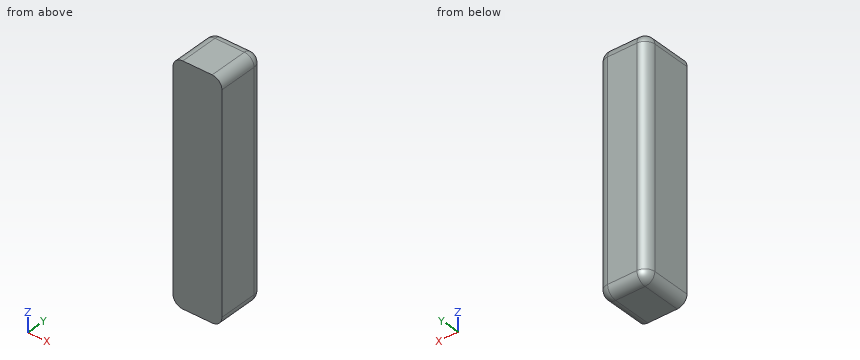
from build123d import *

# Parameters (mm, degrees)
SKETCH_1_W          = 50
SKETCH_1_H          = 50
EXTRUDE_2_DEPTH     = 240
EXTRUDE_3_DEPTH     = 5
FILLET_1_R          = 10
SKETCH_3_W          = 340
SKETCH_3_H          = 5
CUT_EXTRUDE_1_DEPTH = 59


with BuildPart() as part:
    # 草图1 → 凸台-拉伸2 (new body)
    with BuildSketch(Plane.XY):
        with Locations((25, 25)):
            Rectangle(SKETCH_1_W, SKETCH_1_H)
    extrude(amount=EXTRUDE_2_DEPTH)

    # 草图2 → 凸台-拉伸3 (add)
    with BuildSketch(Plane.XZ):
        Polygon((0, 240), (0, 290), (50, 290), (50, 0), (50, -50), (0, -50), align=None)
    extrude(amount=EXTRUDE_3_DEPTH)

    # 圆角1
    fillet_1_edges = [part.edges().sort_by_distance(p)[0] for p in [
        (25, 50, 240),
        (0, 25, 240),
        (50, 25, 240),
        (50, 50, 120),
        (50, 25, 0),
        (0, 25, 0),
        (25, 50, 0),
        (0, 50, 120),
    ]]
    fillet(fillet_1_edges, radius=FILLET_1_R)

    # 草图3 → 切除-拉伸1 (cut)
    with BuildSketch(Plane.ZY):
        with Locations((120, -2.5)):
            Rectangle(SKETCH_3_W, SKETCH_3_H)
    extrude(amount=-CUT_EXTRUDE_1_DEPTH, mode=Mode.SUBTRACT)


solid = part.part
Geometry check sheet. Reference: the model listing, model coordinates, mm. Give positions to 0.01 mm unless a question says otherwise; leave off trailing zeros. Order: outer loops, then holes, each group sorted by start corner. A loop starts at its lowest first (then second) coordinate and runs counter-clockwise, first axis right, second up.
1) Cross-section at A-A (z = 191.5). Record the boundary of the cut face in (x, y).
Results are:
outline: (0, 0) - (50, 0) - (50, 40) arc R10 ccw to (40, 50) - (10, 50) arc R10 ccw to (0, 40) - close
2) Gauge pin test, flat end, axial feed: pin 1 (1 mm diameter, centred on x = 8.5, y = 12.5, fed in from -Z). Record the tip position at first contact, or that the pin passes through.
Results are:
pin 1: stops at z = 0.05
3) Cross-section at C-C (x = 5). Record the boundary of the cut face in (y, z).
Results are:
outline: (0, 1.34) - (40, 1.34) arc R8.66 ccw to (48.66, 10) - (48.66, 230) arc R8.66 ccw to (40, 238.66) - (0, 238.66) - close
4) Material ranges on probe 1 along Z at (x, y) = (7, 39.5); probe 2 along Y at (x, z) = (4.5, 132.5); probe 3 along X at (y, z) = (41.5, 184.5), recorded low to high.
Results are:
probe 1: z = 0.46 to 239.54
probe 2: y = 0 to 48.35
probe 3: x = 0.11 to 49.89
5) Cross-section at B-B (y = 44). Record the boundary of the cut face in (x, z).
Results are:
outline: (0.83, 10) arc R9.17 ccw to (10, 0.83) - (40, 0.83) arc R9.17 ccw to (49.17, 10) - (49.17, 230) arc R9.17 ccw to (40, 239.17) - (10, 239.17) arc R9.17 ccw to (0.83, 230) - close
